Source: CAD feature listing. Evaluate the final solid. Frame: model axes, mm. A direction names the side the tool comes from. Give positions to 0.01 mm unless a question says otherwise; leave off trailing zeros. Order: outer loops, then holes, each group sorted by start corner. A loop starts at its lowest first (then second) coordinate and runs counter-clockwise, first axis right, second up. Notation, with made-up numbers: M 57.5,32 L 80.5,32 A21 cw 80.5,64 Z; hole C 39.5,-33 d7. An arc over 180 degrees is marked long. Answer as a JSON object with one key per item and string values. Group by question number.
1. Pin query (flat end, axial travel): P1, Ø12, axis at y = 1483, z = 28.5, coming from the +X side; P2, Ø8, axis at y = 1196.5, z = 31, coming from the -X side; P3, Ø2, axis at y = 221, z = 24.5, coming from the -X side. Return the tip coordinate at first contact, or that it passes through.
2. Section query A-A (z = 8). Output: boundary loops of the cut face in (x, y), plus the area to 3 significant figures.
3. Section query B-B (x = 117.5). Output: boundary loops of the cut face in (y, z), plus the area to 3 significant figures.
4. Material intervals for L1, parallel to Y at x = 82, z = 13; L2, parallel to X at y = 650, z = 32; L3, parallel to Y at x = 111.5, z = 29, sorted ascending. Write a range as [from, to].
5. Section query C-C (y = 1178). Output: boundary loops of the cut face in (x, z).
6. Set-up query: faces 1 (the flat face through (215, 720, 20)), 2 (the flat face through (0, 557, 20)), 3 (the flat face through (139, 1420, 20)). Return all of +Z, -Z, +X, -X, +Y, -Y with unobstructed straight access to the full face (end or side cutting, diameter ignored); none if empty.
from build123d import *

# Parameters (mm, degrees)
SKETCH1_R           = 9
BOSS_EXTRUDE1_DEPTH = 40
M24_TAPPED_HOLE1_D  = 21
FILLET1_R           = 15
FILLET2_R           = 10


with BuildPart() as part:
    # Sketch1 → Boss-Extrude1 (new body)
    with BuildSketch(Plane.XY):
        Polygon((0, 0), (0, 1145.516137583), (-33.72387302, 1145.516137583), (-80.68, 1300), (-80.68, 1520), (55, 1520), (55, 1420), (215, 1420), (215, 0), align=None)
        with Locations((26, 251)):
            Circle(SKETCH1_R, mode=Mode.SUBTRACT)
        with Locations((26, 651)):
            Circle(SKETCH1_R, mode=Mode.SUBTRACT)
    extrude(amount=BOSS_EXTRUDE1_DEPTH)

    # M24 Tapped Hole1 (through all)
    with Locations(Plane(origin=(18.132788177, 1250, 0), x_dir=(-1, 0, 0), z_dir=(0, 0, -1))):
        with Locations((0, 0), (-63.867211823, -600), (-63.867211823, -1090)):
            Hole(M24_TAPPED_HOLE1_D / 2)

    # Fillet1
    fillet1_edges = [part.edges().sort_by_distance(p)[0] for p in [
        (0, 1145.516137583, 20),
        (-33.72387302, 1145.516137583, 20),
    ]]
    fillet(fillet1_edges, radius=FILLET1_R)

    # Fillet2
    fillet2_edges = [part.edges().sort_by_distance(p)[0] for p in [
        (-80.68, 1520, 20),
        (55, 1520, 20),
        (55, 1420, 20),
    ]]
    fillet(fillet2_edges, radius=FILLET2_R)


solid = part.part
Answer sheet:
{
 "1": {"P1": "x = 55", "P2": "x = -50.44", "P3": "x = 0"},
 "2": {"outline": "M -80.68,1300 L -36.96,1156.15 A15 ccw -22.61,1145.52 L -15,1145.52 A15 cw 0,1130.52 L 0,0 L 215,0 L 215,1420 L 65,1420 A10 cw 55,1430 L 55,1510 A10 ccw 45,1520 L -70.68,1520 A10 ccw -80.68,1510 Z; hole C 18.13,1250 d21; hole C 26,251 d18; hole C 26,651 d18; hole C 82,160 d21; hole C 82,650 d21", "area": "336,000 mm^2"},
 "3": {"outline": "M 0,0 L 1420,0 L 1420,40 L 0,40 Z", "area": "56,800 mm^2"},
 "4": {"L1": "[0, 149.5], [170.5, 639.5], [660.5, 1420]", "L2": "[0, 17.06], [34.94, 71.5], [92.5, 215]", "L3": "[0, 1420]"},
 "5": {"outline": "M -43.6,0 L 215,0 L 215,40 L -43.6,40 Z"},
 "6": {"face 1": "+Z, -Z, +X, +Y, -Y", "face 2": "+Z, -Z, -X, -Y", "face 3": "+Z, -Z, +X, +Y"}
}
